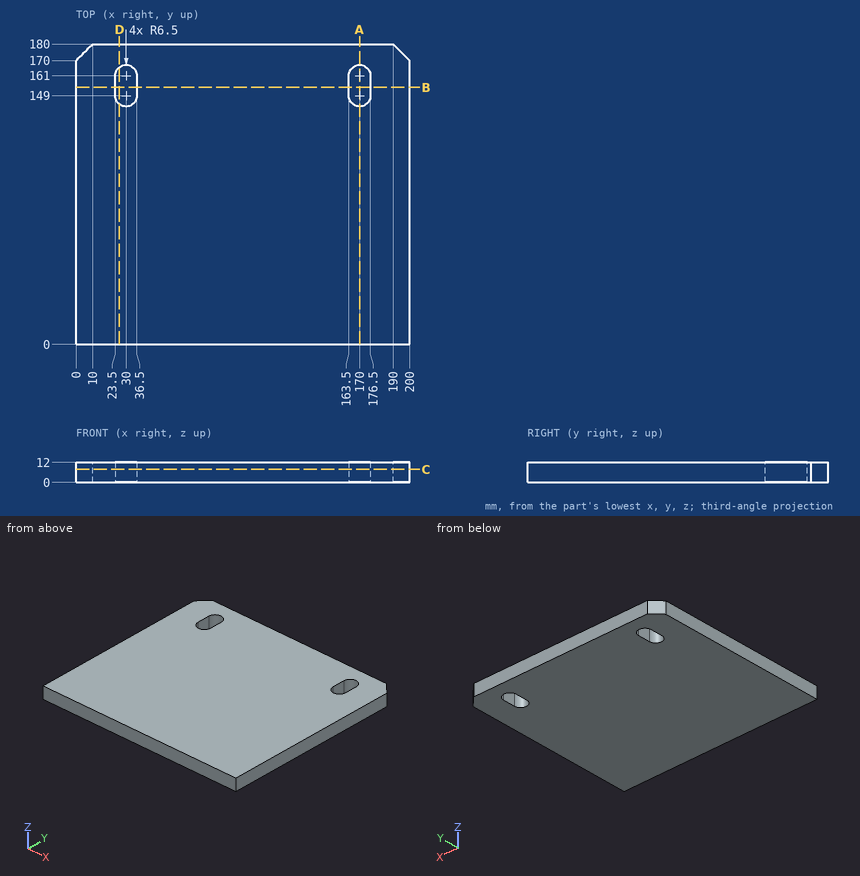
Geometry check sheet. Reference: drawing and pictorial views, mm from the part's lowest x, y, z. Coordinates: 2 decimals unless noted, no trailing zeros. Loops run counter-clockwise (first coordinate to the right, second up) from the corner with the lowest first, then second, coordinate; pieces in that order, holes last. Notation, with made-up numbers: (-15.5, -10) -> (37.5, -10) arc R33 ccw to (37.5, 22) -> close; hole circle Ø10 at (-8, 15.5). An arc over 180 degrees is marked (long way). Write item = value, one per line. Start each with the question number.
1. Section check A-A on x = 170. Record the cut outline in (y, z).
2. Section check B-B on y = 154. Record the cut outline in (x, z).
3. Section check C-C on z = 7.75. Record the cut outline in (x, y).
4. Section check D-D on x = 26. Record the cut outline in (y, z), then the cut area to 3 significant figures.
5. Material ranges on line 1 (X direction, y = 148.5, z = 2.5); line 2 (Y direction, x = 164.5, z = 2.25); line 3 (Y direction, x = 26, z = 1.25), recorded low to high.
Responses:
q1.outline = (0, 0) -> (142.5, 0) -> (142.5, 12) -> (0, 12) -> close; (167.5, 0) -> (180, 0) -> (180, 12) -> (167.5, 12) -> close
q2.outline = (0, 0) -> (23.5, 0) -> (23.5, 12) -> (0, 12) -> close; (36.5, 0) -> (163.5, 0) -> (163.5, 12) -> (36.5, 12) -> close; (176.5, 0) -> (200, 0) -> (200, 12) -> (176.5, 12) -> close
q3.outline = (0, 0) -> (200, 0) -> (200, 170) -> (190, 180) -> (10, 180) -> (0, 170) -> close; hole (23.5, 149) arc R6.5 ccw to (36.5, 149) -> (36.5, 161) arc R6.5 ccw to (23.5, 161) -> close; hole (163.5, 149) arc R6.5 ccw to (176.5, 149) -> (176.5, 161) arc R6.5 ccw to (163.5, 161) -> close
q4.outline = (0, 0) -> (143.88, 0) -> (143.88, 12) -> (0, 12) -> close; (166.12, 0) -> (180, 0) -> (180, 12) -> (166.12, 12) -> close
q4.area = 1,890 mm2
q5.line_1 = 0 to 23.52, 36.48 to 163.52, 176.48 to 200
q5.line_2 = 0 to 145.54, 164.46 to 180
q5.line_3 = 0 to 143.88, 166.12 to 180
